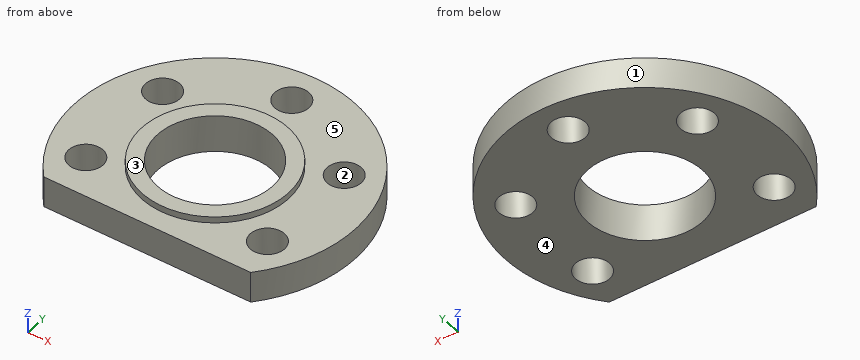
```python
from build123d import *

# Parameters (mm, degrees)
SKETCH_1_R          = 45
SKETCH_1_R_2        = 18.5
EXTRUDE_1_DEPTH     = 10
SKETCH_2_R          = 23.5
SKETCH_2_R_2        = 18.5
EXTRUDE_2_DEPTH     = 2
SKETCH_3_R          = 5.5
CUT_EXTRUDE_1_DEPTH = 65.420493634
CUT_EXTRUDE_2_DEPTH = 65.420493634


with BuildPart() as part:
    # 草图1 → 拉伸1 (new body)
    with BuildSketch(Plane.XY):
        Circle(SKETCH_1_R)
        Circle(SKETCH_1_R_2, mode=Mode.SUBTRACT)
    extrude(amount=EXTRUDE_1_DEPTH)

    # 草图2 → 拉伸2 (add)
    with BuildSketch(Plane.XY.offset(10)):
        Circle(SKETCH_2_R)
        Circle(SKETCH_2_R_2, mode=Mode.SUBTRACT)
    extrude(amount=EXTRUDE_2_DEPTH)

    # 草图3 → 切除-拉伸1 (cut, through all)
    with BuildSketch(Plane.XY.offset(10)):
        with Locations((0, 34)):
            Circle(SKETCH_3_R)
        with Locations((-29.444863729, 17)):
            Circle(SKETCH_3_R)
        with Locations((-29.444863729, -17)):
            Circle(SKETCH_3_R)
        with Locations((29.444863729, 17)):
            Circle(SKETCH_3_R)
        with Locations((29.444863729, -17)):
            Circle(SKETCH_3_R)
    extrude(amount=-CUT_EXTRUDE_1_DEPTH, mode=Mode.SUBTRACT)

    # 草图4 → 切除-拉伸2 (cut, through all)
    with BuildSketch(Plane.XY.offset(10)):
        with BuildLine():
            Line((-35.388711425, -30), (35.388711425, -30))
            ThreePointArc((35.388711425, -30), (0, -46.393543692), (-35.388711425, -30))
        make_face()
    extrude(amount=-CUT_EXTRUDE_2_DEPTH, mode=Mode.SUBTRACT)


solid = part.part
```
Can you work these out from the model? Positions are in its coordinate system, mm. Face numbers are marked on the shaded views. A direction names the side the tool comes from. Coordinates: 2 decimals unless noted, no trailing zeros. Write each loop counter-clockwise with the first axis right and the second up, starting at its lowest first coordinate (ties: lowest second). Pieces come first, ordered by that corner, then holes. Notation, with made-up numbers: M 42,21.25 L 55,21.25 A26 ccw 55,54.25 Z; hole C 42.25,-39 d9. An arc over 180 degrees is marked long. Answer as CSV lines item,"result".
Item 1: Please list where these lines run through material, in increasing order: line 1 along Y through (x, z) = (0, 8); line 2 along Z through (x, y) = (-13, -20); line 3 along X through (y, z) = (0.5, 11).
Geometry results:
line 1,"y = -30 to -18.5, 18.5 to 28.5, 39.5 to 45"
line 2,"z = 0 to 10"
line 3,"x = -23.49 to -18.49, 18.49 to 23.49"
Item 2: Imagine slicing it at B-B on z = 7.75. List the corners of the cut face in (x, y) for me, plus the area to 3 significant figures.
Geometry results:
outline,"M -33.54,-30 L 33.54,-30 A45 ccw long Z; hole C -29.44,-17 d11; hole C -29.44,17 d11; hole C 0,0 d37; hole C 0,34 d11; hole C 29.44,-17 d11; hole C 29.44,17 d11"
area,"4,110 mm2"
Item 3: Imagine slicing it at C-C on y = 34. List the corners of the cut face in (x, z) for me, plus the area to 3 significant figures.
Geometry results:
outline,"M -29.48,0 L -5.5,0 L -5.5,10 L -29.48,10 Z; M 5.5,0 L 29.48,0 L 29.48,10 L 5.5,10 Z"
area,"480 mm2"
Item 4: On a 3-axis mill with a long thin cutter (end or side, diameter ignored), from which of +Z, -Z, +X, -X, +Y, -Y can I reach the whole of each face in a straight line? I mean the marked faces 4 and 5. Say none if no direction works.
Geometry results:
face 4,"-Z, +X, -X, +Y, -Y"
face 5,"+Z"
Item 5: I'm going to push flat-ended pins straight in: P1, Ø9, axis at x = -29.44, y = -17, coming from the -Z side; P2, Ø3, axis at y = 26, z = 10, coming from the +X side; P3, Ø17.5, axis at x = 0, y = 34, coming from the +Z side; P4, Ø6, axis at y = -10.5, z = 8.5, coming from the +X side. Where does each tip first touch, or does it pass through?
Geometry results:
P1,"passes through"
P2,"stops at x = 37.75"
P3,"stops at z = 10"
P4,"stops at x = 44.37"
Item 6: Imagine slicing it at D-D on x = -11. List the corners of the cut face in (y, z) for me.
Geometry results:
outline,"M -30,0 L -14.87,0 L -14.87,12 L -20.77,12 L -20.77,10 L -30,10 Z; M 14.87,0 L 43.63,0 L 43.63,10 L 20.77,10 L 20.77,12 L 14.87,12 Z"
Item 7: Imagine slicing it at A-A on x = 0. List the corners of the cut face in (y, z) for me.
Geometry results:
outline,"M -30,0 L -18.5,0 L -18.5,12 L -23.5,12 L -23.5,10 L -30,10 Z; M 18.5,0 L 28.5,0 L 28.5,10 L 23.5,10 L 23.5,12 L 18.5,12 Z; M 39.5,0 L 45,0 L 45,10 L 39.5,10 Z"
Item 8: We'd pull the mould along Y, two halves only. Please class the marked faces 1, 2 and 3: +Y half, -Y half, draft (parallel to the pull), parting line (faces both ways), or undercut.
Geometry results:
face 1,"parting line"
face 2,"undercut"
face 3,"draft"
